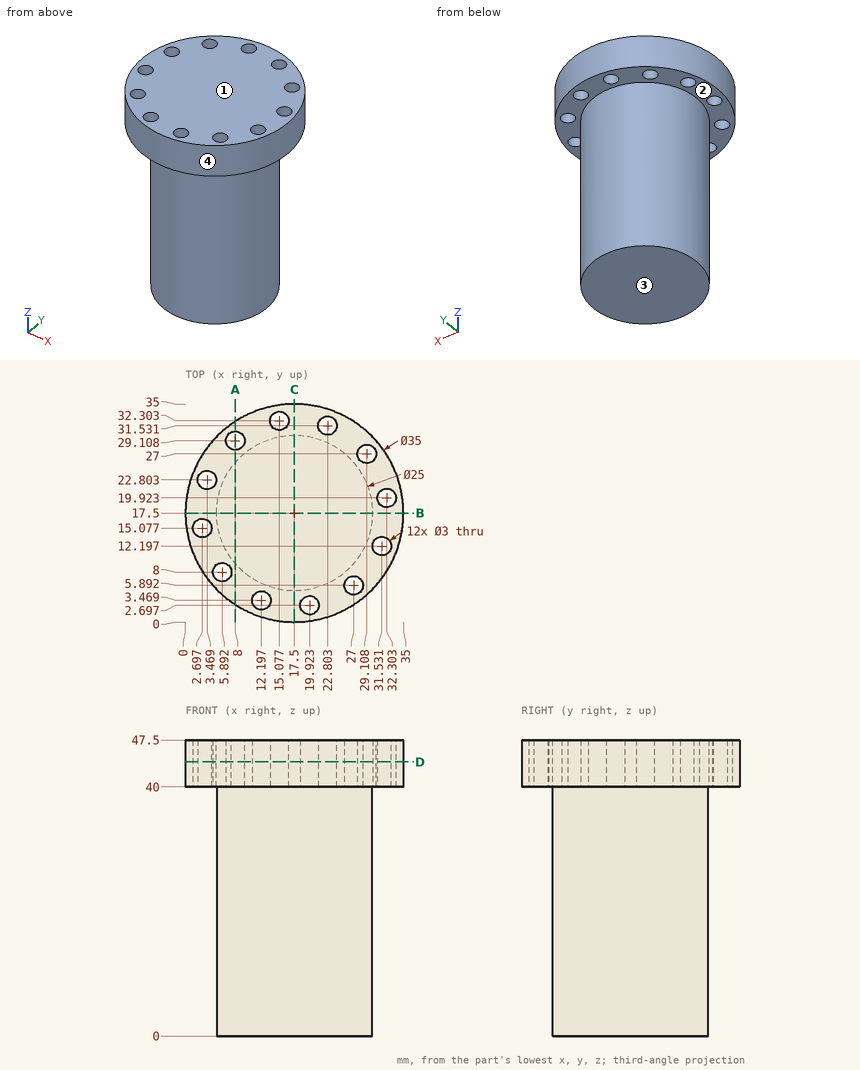
Input: dimensioned drawing with shaded views. Units: mm. Origin: part minimum x, y, z. A direction names the side the tool comes from. Give positions to 0.01 mm unless a question says otherwise; leave off trailing zeros. Loops run counter-clockwise (first coordinate to the right, second up) from the corner with the lowest first, then second, coordinate; pieces in that order, holes last. Notation, with made-up numbers: M 84,11.5 L 112,11.5 A30 cw 112,41.5 Z; hole C -9,26.25 d11. An arc over 180 degrees is marked long. Put each result on its own line as item: value. Start each with the question number.
1) Cut plane D-D (z = 44). Give the number of separate pieces and of enclosed holes in the cut face, then the cut area to 3 significant figures.
2) Cut plane A-A (x = 8). Output: boundary loops of the cut face in (y, z).
3) Contact query for flat-ended pins moving along their axis: pin 1 (4 mm diameter, centred on x = 15.08, y = 32.3, fed in from -Z); pin 2 (1.5 mm diameter, centred on y = 24, z = 27, fed in from +X); pin 3 (3 mm diameter, centred on y = 22, z = 34.5, fed in from -X) (1 decimal); pin 4 (2.5 mm diameter, centred on x = 27, y = 5.89, fed in from -Z). Output: stop coordinate, or through.
4) Cut plane B-B (y = 17.5). Output: boundary loops of the cut face in (x, z).
5) Pull-direction query (Y, two-part tool) for the marked faces 3 and 4; classes: pulls with the +Y half, pulls with the -Y half, needs draft (parallel to the pull), parting line crosses it, or undercut.
6) Access query for the marked faces 1 and 2. Directions: +Z, -Z, +X, -X, +Y, -Y. A direction counts if a zero-diameter tool reaches every point of the face in a straight line with its end or side. Return the directions, or none.
7) Ray query, line 1 along X through (y, z) = (5, 45) (1 decimal); line 2 along X through (y, z) = (17, 33.5); line 3 along Y through (x, z) = (17.5, 20.5). Return the intervals inside material, ascending.
Verdict:
1. separate pieces: 1
1. enclosed holes: 12
1. area: 877 mm2
2. outline: M 2.8,40 L 9.38,40 L 9.38,0 L 25.62,0 L 25.62,40 L 27.61,40 L 27.61,47.5 L 2.8,47.5 Z; M 30.61,40 L 32.2,40 L 32.2,47.5 L 30.61,47.5 Z
3. pin 1: z = 40
3. pin 2: x = 28.6
3. pin 3: x = 5.4
3. pin 4: through
4. outline: M 0,40 L 5,40 L 5,0 L 30,0 L 30,40 L 35,40 L 35,47.5 L 0,47.5 Z
5. face 3: needs draft
5. face 4: parting line crosses it
6. face 1: +Z, +X, -X, +Y, -Y
6. face 2: -Z
7. line 1: 5.3 to 25.8, 28.2 to 29.7
7. line 2: 5.01 to 29.99
7. line 3: 5 to 30
